Verification items for this drawing (mm, ordinates from the low corner). Round coordinates to 2 decimals unless told otherwise and drop trailing zeros. Write each loop counter-clockwise with the first axis right and the second up, starting at its lowest first coordinate (ties: lowest second). Pieces come first, ordered by that corner, then holes. Notation, with made-up numbers: (41, -13) -> (59, -13) arc R24 cw to (59, 25) -> close; hole circle Ø2 at (44.5, 64.25). An arc over 180 degrees is marked (long way). One line per item, written item: value.
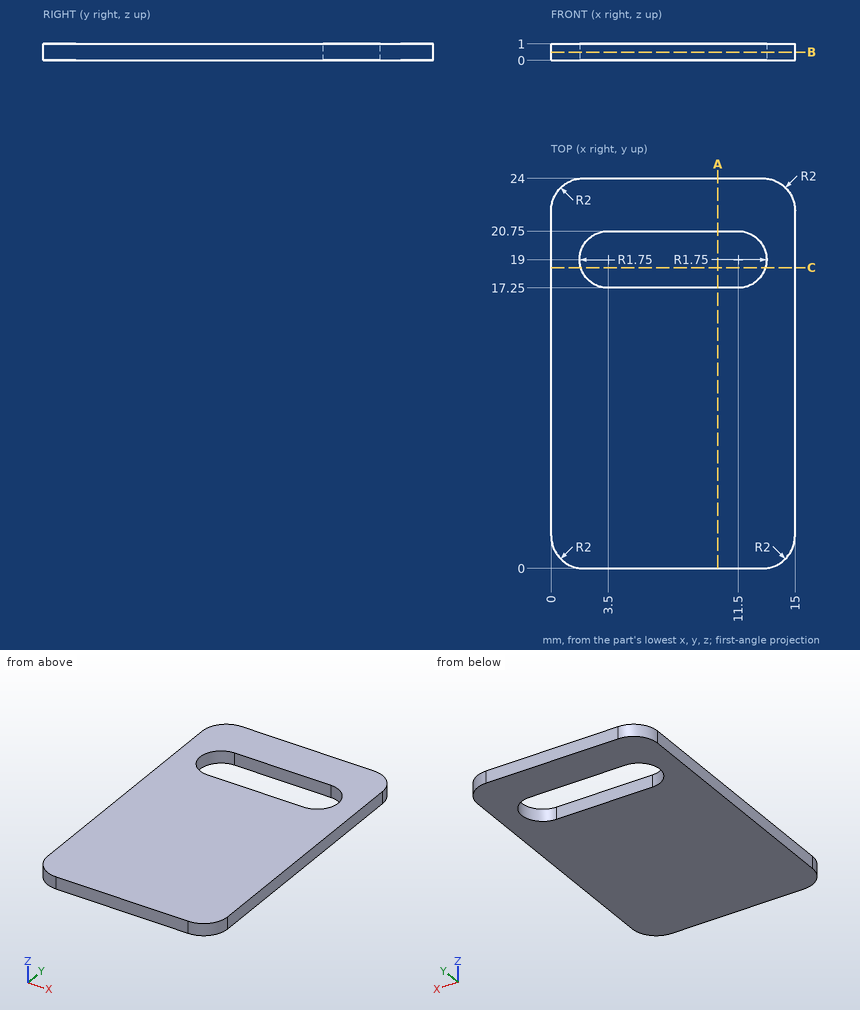
Item 1: Material ranges on line 1 along Y through (x, z) = (9.5, 0.45); line 2 along Y through (x, z) = (12.5, 0.45); line 3 along X through (y, z) = (18.25, 0.95), recorded low to high.
Result set:
line 1: 0 to 17.25, 20.75 to 24
line 2: 0 to 17.56, 20.44 to 24
line 3: 0 to 1.92, 13.08 to 15
Item 2: Sectioned sample at B-B (z = 0.5). Enter the section's corners in (x, y), then the cut area to 3 significant figures.
Result set:
outline: (0, 2) arc R2 ccw to (2, 0) -> (13, 0) arc R2 ccw to (15, 2) -> (15, 22) arc R2 ccw to (13, 24) -> (2, 24) arc R2 ccw to (0, 22) -> close; hole (3.5, 17.25) -> (11.5, 17.25) arc R1.75 ccw to (11.5, 20.75) -> (3.5, 20.75) arc R1.75 ccw to start
area: 319 mm^2
Item 3: Sectioned sample at C-C (y = 18.5). Enter the section's corners in (x, z), then the cut area to 3 significant figures.
Result set:
outline: (0, 0) -> (1.82, 0) -> (1.82, 1) -> (0, 1) -> close; (13.18, 0) -> (15, 0) -> (15, 1) -> (13.18, 1) -> close
area: 3.65 mm^2
Item 4: Sectioned sample at A-A (x = 10.25). Enter the section's corners in (y, z).
Result set:
outline: (0, 0) -> (17.25, 0) -> (17.25, 1) -> (0, 1) -> close; (20.75, 0) -> (24, 0) -> (24, 1) -> (20.75, 1) -> close
